For this review, use the dimensioned drawing (mm, ordinates from the lowest corner) and the shaded views. Give positions to 0.01 mm unless a question says otherwise; leave off trailing zeros. Write each loop counter-clockwise with the first axis right and the second up, starting at its lowest first coordinate (ties: lowest second). Pieces come first, ordered by that corner, then holes.
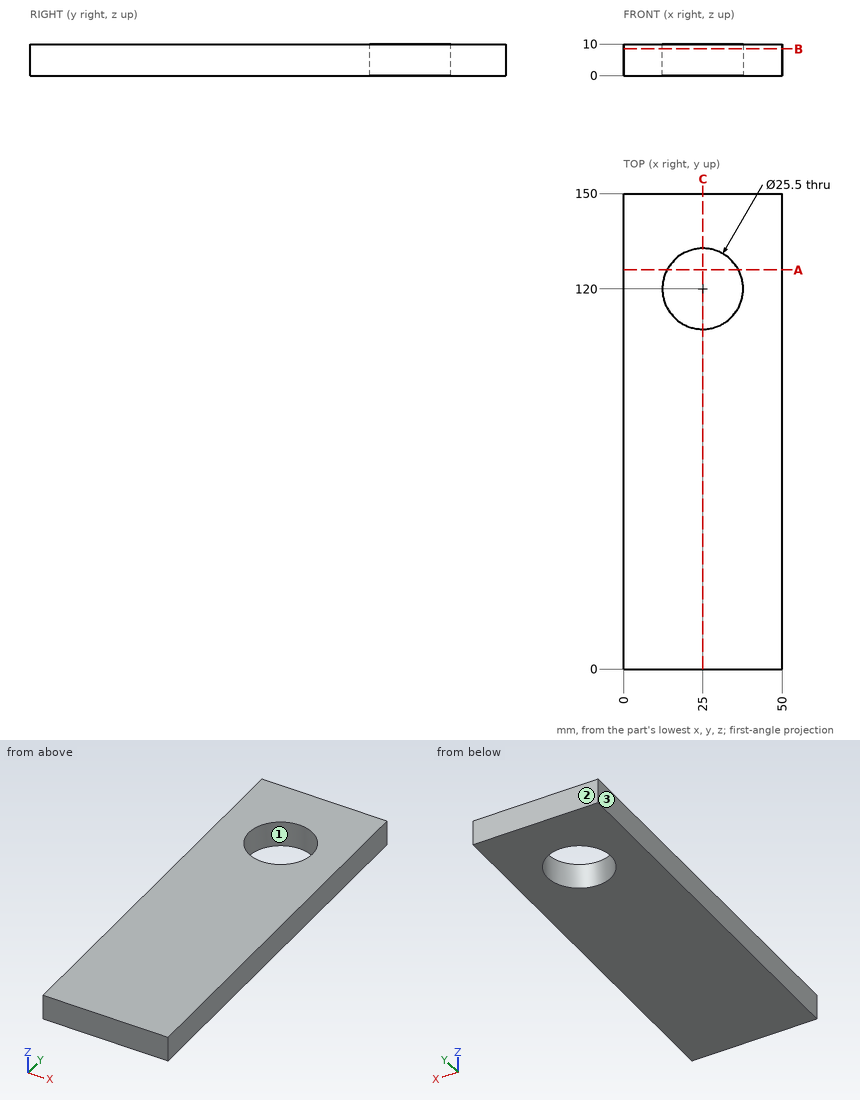
(1) We need section A-A (y = 126). Write out the cut boundary in (x, z).
(2) We need section C-C (x = 25). Write out the cut boundary in (y, z).
(3) The part is to be moulded in two halves that separate along Y. For the marked faces 1, 2 and 3, say which applies: +Y half, -Y half, draft (parallel to the pull), parting line (faces both ways), or undercut.
(4) We need section B-B (z = 8.5). Write out the cut boundary in (x, y), and give its area (3 significant figures).
(5) Clearance check with a flat-ended pin moving along its axis: pin 1 Ø15.5 at (x, y) = (25, 120) entering from -Z. State where the tip first meets the part, or that it passes through.
(6) For L1, parallel to Y at x = 25, z = 6.25; L2, parallel to X at y = 120.5, z = 0.5; L3, parallel to Y at x = 20, z = 6, list the stretches that pass through material, from the lowest coordinate up.
The answers:
1. outline: (0, 0) - (13.75, 0) - (13.75, 10) - (0, 10) - close; (36.25, 0) - (50, 0) - (50, 10) - (36.25, 10) - close
2. outline: (0, 0) - (107.25, 0) - (107.25, 10) - (0, 10) - close; (132.75, 0) - (150, 0) - (150, 10) - (132.75, 10) - close
3. face 1: undercut
3. face 2: +Y half
3. face 3: draft
4. outline: (0, 0) - (50, 0) - (50, 150) - (0, 150) - close; hole circle Ø25.5 at (25, 120)
4. area: 6,990 mm2
5. pin 1: passes through
6. L1: y = 0 to 107.25, 132.75 to 150
6. L2: x = 0 to 12.26, 37.74 to 50
6. L3: y = 0 to 108.27, 131.73 to 150
